Geometry check sheet. Reference: the model listing, model coordinates, mm. Round coordinates to 2 decimals unless told otherwise and drop trailing zeros. Write each loop counter-clockwise with the first axis right and the second up, starting at its lowest first coordinate (ties: lowest second). Pieces come first, ordered by that corner, then holes. Notation, with made-up numbers: M -37.5,22 L -13.5,22 A15 ccw -13.5,46 Z; hole C 31,-27 d6. An arc over 180 degrees is marked long. One line per item, written item: value. Start each with the question number.
1. Section check B-B (y = -50). Record the boundary of the cut face in (x, z), and give its area (3 significant figures).
2. Release check for a two-part mould opening along X. For faces 1 (the flat face through (72, 58, 10)), 2 (the flat face through (1, -60, 10)), 3 (the cylindrical face through (62.63, -57.32, 10.14)) record: pulls with the +X half, pulls with the -X half, needs draft (parallel to the pull), parting line crosses it, or undercut.
3. Section check C-C (x = -61). Record the boundary of the cut face in (y, z), and give its area (3 significant figures).
4. Section check D-D (y = 0). Record the boundary of the cut face in (x, z), and give its area (3 significant figures).
5. Section check A-A (x = 0). Record the boundary of the cut face in (y, z), and give its area (3 significant figures).
6. Scan lines: probe 1 along X at (y, z) = (-50, 4.75); probe 2 along Y at (x, z) = (-61, 10.25); probe 3 along X at (y, z) = (-52, 1.25). Record each from-to range of solid material in increasing order. Write a range as [from, to].
7. Depth check by flat-ended pin: P1, Ø9, axis at x = 61, y = 50, coming from the -Z side. Enter the tip coordinate at first touch or a pass-through.
from build123d import *

# Parameters (mm, degrees)
BOSS_EXTRUDE1_DEPTH     = 20
CUT_EXTRUDE1_DEPTH      = 99.107084352
CUT_EXTRUDE1_DEPTH_BACK = 99.107084352
SKETCH3_R               = 7.5
SKETCH4_R               = 10
CUT_EXTRUDE2_DEPTH      = 59
CUT_EXTRUDE3_REACH      = 100.107
SKETCH5_R               = 6


with BuildPart() as part:
    # Sketch2 → Boss-Extrude1 (new body)
    with BuildSketch(Plane.XY):
        Polygon((75, -55), (70, -60), (-70, -60), (-75, -55), (-75, 55), (-70, 60), (70, 60), (75, 55), align=None)
    extrude(amount=BOSS_EXTRUDE1_DEPTH)

    # Sketch3 → Cut-Extrude1 (cut, two sides: drawn at the far end of the back side and taken through both)
    with BuildSketch(Plane(origin=(0, 0, 0), x_dir=(-1, 0, 0), z_dir=(0, 0, -1)).offset(-CUT_EXTRUDE1_DEPTH_BACK)):
        with Locations((61, -50)):
            Circle(SKETCH3_R)
        with Locations((61, 50)):
            Circle(SKETCH3_R)
        with Locations((-61, -50)):
            Circle(SKETCH3_R)
        with Locations((-61, 50)):
            Circle(SKETCH3_R)
    extrude(amount=CUT_EXTRUDE1_DEPTH + CUT_EXTRUDE1_DEPTH_BACK, mode=Mode.SUBTRACT)

    # Sketch4 → Cut-Extrude2 (cut)
    with BuildSketch(Plane(origin=(0, 0, 0), x_dir=(-1, 0, 0), z_dir=(0, 0, -1))):
        Circle(SKETCH4_R)
    extrude(amount=-CUT_EXTRUDE2_DEPTH, mode=Mode.SUBTRACT)

    # Sketch5 → Cut-Extrude3 (cut, up to next)
    with BuildSketch(Plane(origin=(0, 0, 0), x_dir=(-1, 0, 0), z_dir=(0, 0, -1)), mode=Mode.PRIVATE) as cut_extrude3_sk1:
        with Locations((-16.378850905, -39.542043991)):
            Circle(SKETCH5_R)
    cut_extrude3_tool1 = extrude(cut_extrude3_sk1.sketch, amount=-CUT_EXTRUDE3_REACH, mode=Mode.PRIVATE) & part.part
    # Sketch5 → Cut-Extrude3 (cut, up to next)
    with BuildSketch(Plane(origin=(0, 0, 0), x_dir=(-1, 0, 0), z_dir=(0, 0, -1)), mode=Mode.PRIVATE) as cut_extrude3_sk2:
        with Locations((16.378850905, 39.542043991)):
            Circle(SKETCH5_R)
    cut_extrude3_tool2 = extrude(cut_extrude3_sk2.sketch, amount=-CUT_EXTRUDE3_REACH, mode=Mode.PRIVATE) & part.part
    add(cut_extrude3_tool1.solids().sort_by_distance((16.378851, -39.542044, 0))[0], mode=Mode.SUBTRACT)
    add(cut_extrude3_tool2.solids().sort_by_distance((-16.378851, 39.542044, 0))[0], mode=Mode.SUBTRACT)


solid = part.part
Result sheet:
1. outline: M -75,0 L -68.5,0 L -68.5,20 L -75,20 Z; M -53.5,0 L 53.5,0 L 53.5,20 L -53.5,20 Z; M 68.5,0 L 75,0 L 75,20 L 68.5,20 Z
1. area: 2,400 mm2
2. face 1: pulls with the +X half
2. face 2: needs draft
2. face 3: undercut
3. outline: M -60,0 L -57.5,0 L -57.5,20 L -60,20 Z; M -42.5,0 L 42.5,0 L 42.5,20 L -42.5,20 Z; M 57.5,0 L 60,0 L 60,20 L 57.5,20 Z
3. area: 1,800 mm2
4. outline: M -75,0 L -10,0 L -10,20 L -75,20 Z; M 10,0 L 75,0 L 75,20 L 10,20 Z
4. area: 2,600 mm2
5. outline: M -60,0 L -10,0 L -10,20 L -60,20 Z; M 10,0 L 60,0 L 60,20 L 10,20 Z
5. area: 2,000 mm2
6. probe 1: x = [-75, -68.5], [-53.5, 53.5], [68.5, 75]
6. probe 2: y = [-60, -57.5], [-42.5, 42.5], [57.5, 60]
6. probe 3: x = [-75, -68.23], [-53.77, 53.77], [68.23, 75]
7. P1: passes through
